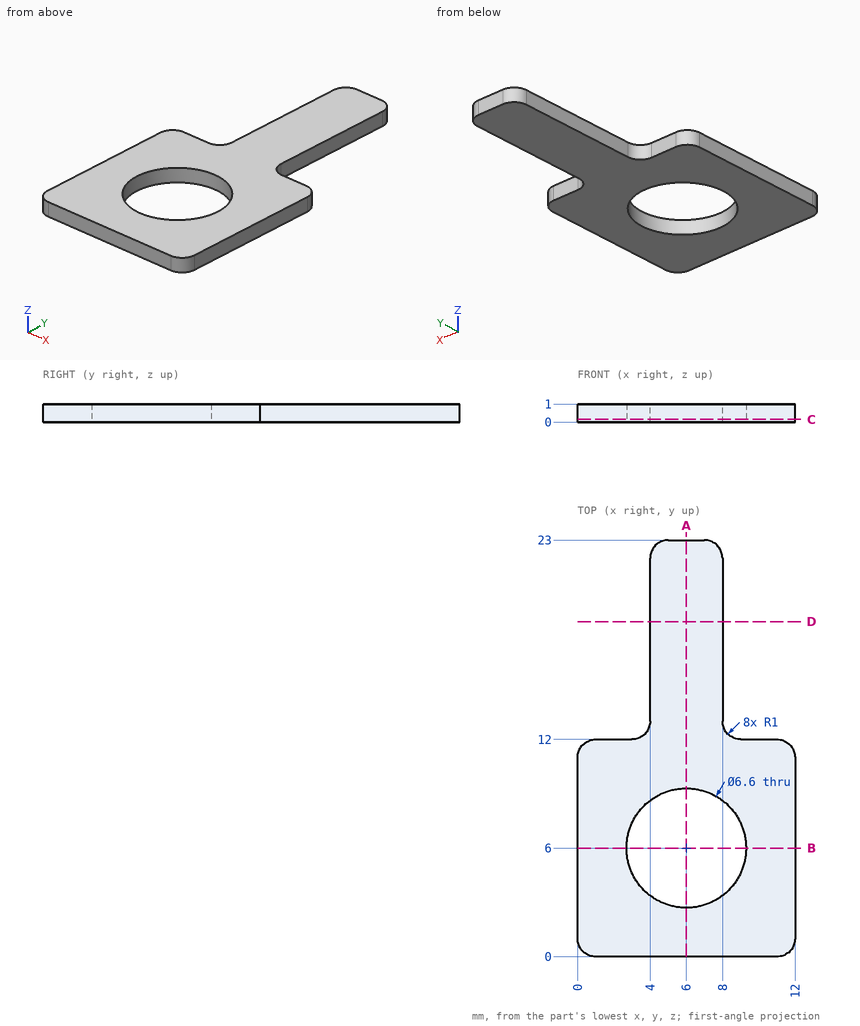
Print and shaded views of the part. All mm, measured from the part's lowest x, y and z. Coordinates: 2 decimals unless noted, no trailing zeros. Order: outer loops, then holes, each group sorted by start corner. A loop starts at its lowest first (then second) coordinate and runs counter-clockwise, first axis right, second up. Notation, with made-up numbers: (19, 59.25) - (43, 59.25) arc R23 ccw to (43, 68.25) - close; hole circle Ø11 at (43.5, 0.5). An arc over 180 degrees is marked (long way). Return JSON: item names as keys, results as strings. Group by question number.
Item 1: Drill centre lines: probe 1 along Y at (x, z) = (6, 0.45); probe 2 along X at (y, z) = (22, 0.9); probe 3 along Y at (x, z) = (2.5, 0.6). Where is each one in solid material? Low to high. Write a range as from..to.
Item 2: Cut at B-B (y = 6). List the corners of the cut face in (x, z), plus the area to 3 significant figures.
Item 3: Cut at C-C (z = 0.15). List the corners of the cut face in (x, y), plus the area to 3 significant figures.
Item 4: Cut at A-A (x = 6). List the corners of the cut face in (y, z), plus the area to 3 significant figures.
Item 5: Cut at D-D (y = 18.5). List the corners of the cut face in (x, z).
Check values:
{
 "1": {"probe 1": "y = 0..2.7, 9.3..23", "probe 2": "x = 4..8", "probe 3": "y = 0..12"},
 "2": {"outline": "(0, 0) - (2.7, 0) - (2.7, 1) - (0, 1) - close; (9.3, 0) - (12, 0) - (12, 1) - (9.3, 1) - close", "area": "5.40 mm2"},
 "3": {"outline": "(0, 1) arc R1 ccw to (1, 0) - (11, 0) arc R1 ccw to (12, 1) - (12, 11) arc R1 ccw to (11, 12) - (9, 12) arc R1 cw to (8, 13) - (8, 22) arc R1 ccw to (7, 23) - (5, 23) arc R1 ccw to (4, 22) - (4, 13) arc R1 cw to (3, 12) - (1, 12) arc R1 ccw to (0, 11) - close; hole circle Ø6.6 at (6, 6)", "area": "153 mm2"},
 "4": {"outline": "(0, 0) - (2.7, 0) - (2.7, 1) - (0, 1) - close; (9.3, 0) - (23, 0) - (23, 1) - (9.3, 1) - close", "area": "16.4 mm2"},
 "5": {"outline": "(4, 0) - (8, 0) - (8, 1) - (4, 1) - close"}
}
